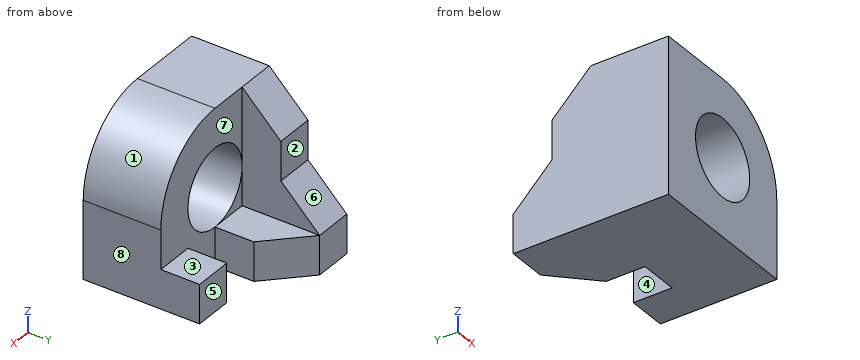
```python
from build123d import *

# Parameters (mm, degrees)
BASE_BLOCK_DEPTH        = 10
CORNER_POST_PROFILE_W   = 10
CORNER_POST_PROFILE_H   = 10
CORNER_POST_10X10_DEPTH = 10
STEPPED_RIB_DEPTH       = 10
GUSSET_DEPTH            = 10
BORE_PROFILE_R          = 10
BORE_20_DEPTH           = 20


with BuildPart() as part:
    # Base Block Profile → Base Block (new, symmetric)
    with BuildSketch(Plane(origin=(0, 0, 0), x_dir=(1, 0, 0), z_dir=(0, 1, 0))):
        with BuildLine():
            Line((0, -20), (-20, -20))
            Line((-20, -20), (-20, 20))
            Line((-20, 20), (20, 20))
            Line((20, 20), (20, 0))
            ThreePointArc((20, 0), (14.142135624, -14.142135624), (0, -20))
        make_face()
    extrude(amount=BASE_BLOCK_DEPTH, both=True)

    # Corner Post Profile → Corner Post 10x10 (add)
    with BuildSketch(Plane(origin=(0, 10, 0), x_dir=(1, 0, 0), z_dir=(0, 1, 0))):
        with Locations((15, 15)):
            Rectangle(CORNER_POST_PROFILE_W, CORNER_POST_PROFILE_H)
    extrude(amount=CORNER_POST_10X10_DEPTH)

    # Stepped Rib Profile → Stepped Rib (add)
    with BuildSketch(Plane.ZY.offset(20)):
        Polygon((-20, 10), (-20, 30), (-10, 30), (0, 20), (10, 20), (20, 10), align=None)
    extrude(amount=-STEPPED_RIB_DEPTH)

    # Gusset Profile → Gusset (add)
    with BuildSketch(Plane(origin=(0, 0, -20), x_dir=(-1, 0, 0), z_dir=(0, 0, -1))):
        Polygon((10, 10), (10, 30), (0, 20), (0, 10), align=None)
    extrude(amount=-GUSSET_DEPTH)

    # Bore Profile → Bore Ø20 (cut)
    with BuildSketch(Plane.XZ.offset(10)):
        with Locations(Location((0, 0, 0), (0, 0, 270))):
            Circle(BORE_PROFILE_R)
    extrude(amount=-BORE_20_DEPTH, mode=Mode.SUBTRACT)


solid = part.part
```
Input: part model. Units: mm. Frame: model coordinates. Face numbers are marked on the shaded views. A direction names the side the tool comes from. Coordinates: 2 decimals unless noted, no trailing zeros. Write each loop counter-clockwise with the first axis right and the second up, starting at its lowest first coordinate (ties: lowest second). Pieces come first, ordered by that corner, then holes. Notation, with made-up numbers: (36, 39.25) -> (64, 39.25) arc R21 cw to (64, 45.25) -> close; hole circle Ø10 at (-28, 58.25). An arc over 180 degrees is marked (long way). Write each question's results on one line, items separated by ' | '.
Item 1: Mould query, pull axis X, two halves, no side actions, for the marked faces 6, 7 and 8. Classes: +X half, -X half, draft (parallel to the pull), parting line (faces both ways), or undercut.
Conclusion:
face 6: draft | face 7: undercut | face 8: +X half
Item 2: Pin query (flat end, axial travel): pin 1 Ø3 at (x, y) = (13, 16.5) entering from +Z; pin 2 Ø8 at (x, z) = (16, -14) entering from +Y; pin 3 Ø8 at (x, z) = (14, -3.5) entering from +Y. Return the tip coordinate at first contact, or that it passes through.
Conclusion:
pin 1: stops at z = -10 | pin 2: stops at y = 20 | pin 3: stops at y = 10
Item 3: Section query D-D on y = 2.5. Return loops of the section in (x, z), plus the area to 3 significant figures.
Conclusion:
outline: (-20, -20) -> (20, -20) -> (20, 0) arc R20 ccw to (0, 20) -> (-20, 20) -> close; hole circle Ø20 at (0, 0) | area: 1,200 mm^2
Item 4: Section query A-A on x = -5. Return loops of the section in (y, z).
Conclusion:
outline: (-10, -20) -> (25, -20) -> (25, -10) -> (10, -10) -> (10, -8.66) -> (-10, -8.66) -> close; (-10, 8.66) -> (10, 8.66) -> (10, 20) -> (-10, 20) -> close
Item 5: Section query C-C on x = -17. Return loops of the section in (y, z).
Conclusion:
outline: (-10, -20) -> (30, -20) -> (30, -10) -> (20, 0) -> (20, 10) -> (10, 20) -> (-10, 20) -> close
Item 6: Section query B-B on z = 7. Return loops of the section in (x, y) (3 decimals).
Conclusion:
outline: (-20, -10) -> (-7.141, -10) -> (-7.141, 10) -> (-10, 10) -> (-10, 20) -> (-20, 20) -> close; (7.141, -10) -> (18.735, -10) -> (18.735, 10) -> (7.141, 10) -> close
Item 7: Set-up query: the marked faces 1, 2, 3, 4 and 5. Return all of +Z, -Z, +X, -X, +Y, -Y with unobstructed straight access to the full face (end or side cutting, diameter ignored); none if empty.
Conclusion:
face 1: +Z, +X, +Y, -Y | face 2: +Z, +X, -X, +Y | face 3: +Z, +X, +Y | face 4: +Z, -Z, +Y | face 5: +Z, -Z, +X, +Y
Item 8: Material intervals for probe 1 along X at (y, z) = (-4.25, 0); probe 2 along Y at (x, z) = (-3.5, 15), sorted ascending.
Conclusion:
probe 1: x = -20 to -10, 10 to 20 | probe 2: y = -10 to 10
